Model file for the job. Use its own axes, mm. A direction names the side the tool comes from. Give positions to 0.01 mm unless a question says otherwise; leave off trailing zeros. Write each loop counter-clockwise with the first axis right and the second up, starting at its lowest first coordinate (ties: lowest second). Pieces come first, ordered by that corner, then holes. Notation, with made-up numbers: (-22.75, 33) - (35.25, 33) arc R19 ccw to (35.25, 57) - close; hole circle Ø1 at (-40, 73.5). An arc over 180 degrees is marked (long way). One line per item, written item: value. Start each with the question number.
(1) Drop flat-ended pins along their axis: P1, Ø1, axis at x = -28.5, z = -19, coming from the -Y side; P2, Ø6.5, axis at x = 54.13, z = -31.25, coming from the +Y side; P3, Ø3, axis at y = 6, z = 25, coming from the -X side. Give the stop position or say it passes through.
(2) Cut at C-C, the plane y = 10. State how many separate pieces and enclosed holes the cut face has, and give its area (3 significant figures).
(3) Cut at B-B, the plane x = 31.75. List the corners of the cut face in (y, z), and give its area (3 significant figures).
(4) Cut at A-A, the plane z = 0. List the corners of the cut face in (x, y), and give its area (3 significant figures).
(5) Mould opens along X. For faces 5 (the face through (-65, 6, 1)), 6 (the face through (52.385, 6.751, -57.395)), 7 (the face through (57.4, 7.69, 23.16)) say: pulls with the +X half, pulls with the -X half, needs draft (parallel to the pull), parting line crosses it, or undercut.
(6) Probe L1, parallel to Z at x = -54, y = 9.5; L2, parallel to Z at x = -57.75, y = 6; L3, parallel to X at y = 6, z = -58.5. List the from-to ranges inside material, lowest first.
(7) 3-axis set-ups, long thin cutter, end or side, ignore diameter. For faces 1 (the face through (-52.385, 6.751, 57.395)), 2 (the face through (-15, 8, 15)), 3 (the face through (-57.4, 7.69, 26.84)), 4 (the face through (-45, 2, 0)): which of +Z, -Z, +X, -X, +Y, -Y reach the whole face in a straight line?
from build123d import *

# Parameters (mm, degrees)
SKETCH_1_W             = 130
SKETCH_1_H             = 130
EXTRUDE_1_DEPTH        = 12
SKETCH_2_R             = 20
CUT_EXTRUDE_1_DEPTH    = 93.703829479
HOLE_WIZARD_M6_1_D     = 7
SKETCH_5_R             = 35
CUT_EXTRUDE_2_DEPTH    = 4
SKETCH_6_R             = 45
CUT_EXTRUDE_3_DEPTH    = 4
HOLE_WIZARD_M6_1_2_D   = 5
HOLE_WIZARD_M6_2_D     = 5
HOLE_WIZARD_M6_2_DEPTH = 15
HOLE_WIZARD_M6_2_TIP   = 1.502151548
HOLE_WIZARD_M6_3_D     = 5
HOLE_WIZARD_M6_3_DEPTH = 15
HOLE_WIZARD_M6_3_TIP   = 1.502151548
HOLE_WIZARD_M6_4_D     = 5
HOLE_WIZARD_M6_4_DEPTH = 15
HOLE_WIZARD_M6_4_TIP   = 1.502151548
HOLE_WIZARD_M6_5_D     = 5
HOLE_WIZARD_M6_5_DEPTH = 15
HOLE_WIZARD_M6_5_TIP   = 1.502151548
CHAMFER_1_SIZE         = 5


with BuildPart() as part:
    # 草图1 → 凸台-拉伸1 (new body)
    with BuildSketch(Plane(origin=(0, 0, 0), x_dir=(1, 0, 0), z_dir=(0, 1, 0))):
        Rectangle(SKETCH_1_W, SKETCH_1_H)
    extrude(amount=EXTRUDE_1_DEPTH)

    # 草图2 → 切除-拉伸1 (cut, through all)
    with BuildSketch(Plane(origin=(0, 12, 0), x_dir=(1, 0, 0), z_dir=(0, 1, 0))):
        with Locations(Location((0, 0, 0), (0, 0, 270))):
            Circle(SKETCH_2_R)
    extrude(amount=-CUT_EXTRUDE_1_DEPTH, mode=Mode.SUBTRACT)

    # Hole Wizard M6 _1 (through all)
    with Locations(Plane(origin=(0, 12, 0), x_dir=(1, 0, 0), z_dir=(0, 1, 0))):
        with Locations((31.250000582, 54.1265874), (54.126588073, 31.249999418), (54.1265874, -31.250000582), (31.249999418, -54.126588073), (-31.250000582, -54.1265874), (-54.126588073, -31.249999418), (-54.1265874, 31.250000582), (-31.249999418, 54.126588073)):
            Hole(HOLE_WIZARD_M6_1_D / 2)

    # 草图5 → 切除-拉伸2 (cut)
    with BuildSketch(Plane(origin=(0, 12, 0), x_dir=(1, 0, 0), z_dir=(0, 1, 0))):
        with Locations(Location((0, 0, 0), (0, 0, 270))):
            Circle(SKETCH_5_R)
    extrude(amount=-CUT_EXTRUDE_2_DEPTH, mode=Mode.SUBTRACT)

    # 草图6 → 切除-拉伸3 (cut)
    with BuildSketch(Plane.XZ):
        with Locations(Location((0, 0, 0), (0, 0, 270))):
            Circle(SKETCH_6_R)
    extrude(amount=-CUT_EXTRUDE_3_DEPTH, mode=Mode.SUBTRACT)

    # Hole Wizard M6 _1 2 (through all)
    with Locations(Plane(origin=(0, 12, 0), x_dir=(1, 0, 0), z_dir=(0, 1, 0))):
        with Locations((-31.75, 31.75), (31.75, 31.75), (31.75, -31.75), (-31.75, -31.75)):
            Hole(HOLE_WIZARD_M6_1_2_D / 2)

    # M6 螺纹孔2
    with Locations(Plane.ZY.offset(65)):
        with Locations((-25, 6), (25, 6)):
            Hole(HOLE_WIZARD_M6_2_D / 2, depth=HOLE_WIZARD_M6_2_DEPTH)
            with Locations((0, 0, -(HOLE_WIZARD_M6_2_DEPTH + HOLE_WIZARD_M6_2_TIP / 2))):  # 118° drill point
                Cone(0, HOLE_WIZARD_M6_2_D / 2, HOLE_WIZARD_M6_2_TIP, mode=Mode.SUBTRACT)

    # M6 螺纹孔3
    with Locations(Plane(origin=(65, 0, 0), x_dir=(0, 0, -1), z_dir=(1, 0, 0))):
        with Locations((-25, 6), (25, 6)):
            Hole(HOLE_WIZARD_M6_3_D / 2, depth=HOLE_WIZARD_M6_3_DEPTH)
            with Locations((0, 0, -(HOLE_WIZARD_M6_3_DEPTH + HOLE_WIZARD_M6_3_TIP / 2))):  # 118° drill point
                Cone(0, HOLE_WIZARD_M6_3_D / 2, HOLE_WIZARD_M6_3_TIP, mode=Mode.SUBTRACT)

    # M6 螺纹孔4
    with Locations(Plane.XY.offset(65)):
        with Locations((-50, 6), (50, 6), (0, 6)):
            Hole(HOLE_WIZARD_M6_4_D / 2, depth=HOLE_WIZARD_M6_4_DEPTH)
            with Locations((0, 0, -(HOLE_WIZARD_M6_4_DEPTH + HOLE_WIZARD_M6_4_TIP / 2))):  # 118° drill point
                Cone(0, HOLE_WIZARD_M6_4_D / 2, HOLE_WIZARD_M6_4_TIP, mode=Mode.SUBTRACT)

    # M6 螺纹孔5
    with Locations(Plane(origin=(0, 0, -65), x_dir=(-1, 0, 0), z_dir=(0, 0, -1))):
        with Locations((-50, 6), (50, 6), (0, 6)):
            Hole(HOLE_WIZARD_M6_5_D / 2, depth=HOLE_WIZARD_M6_5_DEPTH)
            with Locations((0, 0, -(HOLE_WIZARD_M6_5_DEPTH + HOLE_WIZARD_M6_5_TIP / 2))):  # 118° drill point
                Cone(0, HOLE_WIZARD_M6_5_D / 2, HOLE_WIZARD_M6_5_TIP, mode=Mode.SUBTRACT)

    # 倒角1
    chamfer_1_edges = [part.edges().sort_by_distance(p)[0] for p in [
        (65, 6, 65),
        (-65, 6, 65),
        (-65, 6, -65),
        (65, 6, -65),
    ]]
    chamfer(chamfer_1_edges, length=CHAMFER_1_SIZE)


solid = part.part
Answers follow:
1. P1: stops at y = 4
1. P2: passes through
1. P3: stops at x = -49.4
2. separate pieces: 1
2. enclosed holes: 13
2. area: 12,600 mm²
3. outline: (0, -65) - (12, -65) - (12, -57.59) - (0, -57.59) - close; (0, -50.66) - (12, -50.66) - (12, -34.25) - (0, -34.25) - close; (0, 34.25) - (12, 34.25) - (12, 50.66) - (0, 50.66) - close; (0, 57.59) - (12, 57.59) - (12, 65) - (0, 65) - close; (4, -29.25) - (12, -29.25) - (12, -14.73) - (8, -14.73) - (8, 14.73) - (12, 14.73) - (12, 29.25) - (4, 29.25) - close
3. area: 922 mm²
4. outline: (-65, 0) - (-45, 0) - (-45, 4) - (-20, 4) - (-20, 8) - (-35, 8) - (-35, 12) - (-65, 12) - close; (20, 4) - (45, 4) - (45, 0) - (65, 0) - (65, 12) - (35, 12) - (35, 8) - (20, 8) - close
4. area: 760 mm²
5. face 5: pulls with the -X half
5. face 6: undercut
5. face 7: needs draft
6. L1: z = -65 to -34.75, -27.75 to 27.75, 34.75 to 65
6. L2: z = -65 to -27.5, -22.5 to 22.5, 27.5 to 65
6. L3: x = -65 to -52.5, -47.5 to -2.5, 2.5 to 47.5, 52.5 to 65
7. face 1: +Z
7. face 2: +Y
7. face 3: -X
7. face 4: -Y
